Can you work these out from the model? Positions are in its coordinate system, mm. Give positions to 0.01 mm unless a question says otherwise; leave off trailing zeros. Order: outer loops, then holes, each group sorted by start corner. A loop starts at its lowest first (then second) coordinate and runs counter-clockwise, first axis right, second up. Notation, with made-up numbers: (6.25, 7) - (20.25, 7) arc R13 cw to (20.25, 27) - close; hole circle Ø6 at (22, -4). An arc over 180 degrees is marked (long way). One line per question, with ' | ' between items.
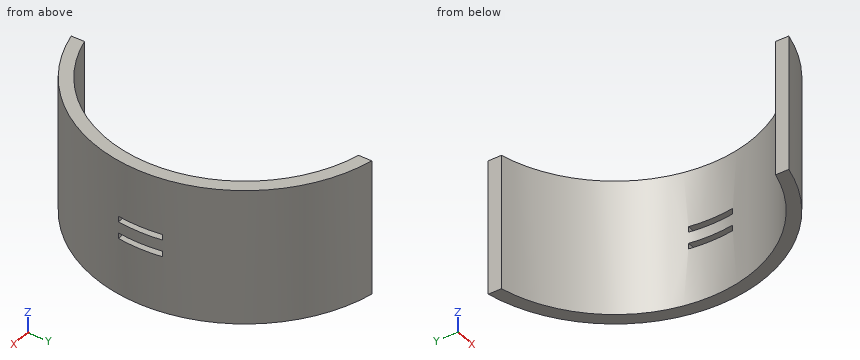
```python
from build123d import *

# Parameters (mm, degrees)
EXTRUDE_1_DEPTH     = 60
SKETCH_3_W          = 2.5
SKETCH_3_H          = 19.1
CUT_EXTRUDE_2_DEPTH = 115


with BuildPart() as part:
    # 草图1 → 凸台-拉伸1 (new body)
    with BuildSketch(Plane.XY):
        with BuildLine():
            Line((15, 65.276254084), (15, 59.535511754))
            ThreePointArc((15, 59.535511754), (61.396067951, 0), (15, -59.535511754))
            Line((15, -59.535511754), (15, -65.276254084))
            ThreePointArc((15, -65.276254084), (66.977528674, 0), (15, 65.276254084))
        make_face()
    extrude(amount=EXTRUDE_1_DEPTH)

    # 草图3 → 切除-拉伸2 (cut)
    with BuildSketch(Plane(origin=(0, 0, 0), x_dir=(0, 0, -1), z_dir=(1, 0, 0))):
        with Locations((-33.75394201, 0)):
            Rectangle(SKETCH_3_W, SKETCH_3_H)
        with Locations((-26.24605799, 0)):
            Rectangle(SKETCH_3_W, SKETCH_3_H)
    extrude(amount=CUT_EXTRUDE_2_DEPTH, mode=Mode.SUBTRACT)


solid = part.part
```
(1) If I drill on line 1 (Z direction, x = 63.5, y = 0); line 2 (Y direction, x = 39, z = 35); line 3 (Y direction, x = 17, z = 45.5), over which ranges is the centre line in solid material (lowest first)?
Answer below:
line 1: 0 to 25, 27.5 to 32.5, 35 to 60 | line 2: -54.45 to -47.42, 47.42 to 54.45 | line 3: -64.78 to -59, 59 to 64.78
(2) Imagine slicing it at C-C (z = 46). List the corners of the cut face in (x, y) for me, and give its area (3 significant figures).
Answer below:
outline: (15, -65.28) arc R66.98 ccw to (15, 65.28) - (15, 59.54) arc R61.4 cw to (15, -59.54) - close | area: 956 mm^2
(3) Imagine slicing it at B-B (y = -6). List the corners of the cut face in (x, z) for me.
Answer below:
outline: (61.1, 0) - (66.71, 0) - (66.71, 25) - (61.1, 25) - close; (61.1, 27.5) - (66.71, 27.5) - (66.71, 32.5) - (61.1, 32.5) - close; (61.1, 35) - (66.71, 35) - (66.71, 60) - (61.1, 60) - close
(4) Imagine slicing it at D-D (x = 32.5). List the corners of the cut face in (y, z) for me, and give its area (3 significant figures).
Answer below:
outline: (-58.56, 0) - (-52.09, 0) - (-52.09, 60) - (-58.56, 60) - close; (52.09, 0) - (58.56, 0) - (58.56, 60) - (52.09, 60) - close | area: 777 mm^2
(5) Will these pins go through, and if not, where does the flat tip stop? pin 1 (5 mm diameter, centred on x = 35, z = 45, fed in from -Y); pin 2 (3 mm diameter, centred on x = 62.5, z = 26.5, fed in from +Y); pin 3 (1 mm diameter, centred on x = 49.5, z = 36, fed in from -Y).
Answer below:
pin 1: y = -58.56 | pin 2: y = 27.66 | pin 3: y = -45.66
(6) Imagine slicing it at A-A (x = 46.5). List the corners of the cut face in (y, z) for me.
Answer below:
outline: (-48.21, 0) - (-40.09, 0) - (-40.09, 60) - (-48.21, 60) - close; (40.09, 0) - (48.21, 0) - (48.21, 60) - (40.09, 60) - close
